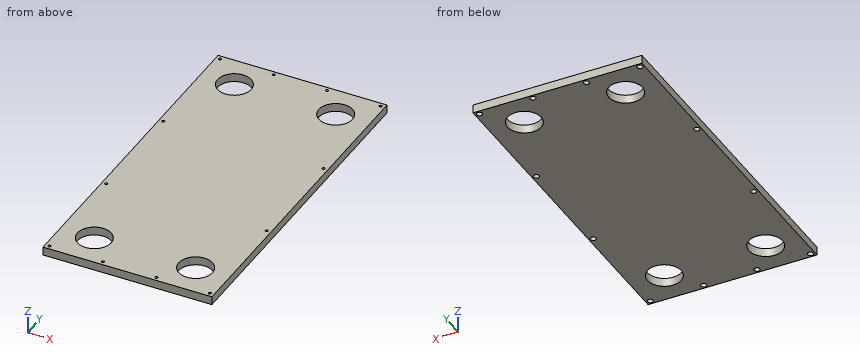
from build123d import *

# Parameters (mm, degrees)
SKETCH1_W                 = 600
SKETCH1_H                 = 1200
BOSS_EXTRUDE1_DEPTH       = 30
SKETCH2_R                 = 60
CUT_EXTRUDE1_DEPTH        = 42
SKETCH3_R                 = 5
CUT_EXTRUDE2_DEPTH        = 40
LPATTERN1_COUNT           = 4
LPATTERN1_PITCH           = 390
LPATTERN2_COUNT           = 2
LPATTERN2_PITCH           = 570
LPATTERN2_COPY_1_SKETCH_R = 5
LPATTERN2_COPY_1_DEPTH    = 40
LPATTERN2_COPY_2_SKETCH_R = 5
LPATTERN2_COPY_2_DEPTH    = 40
LPATTERN2_COPY_3_SKETCH_R = 5
LPATTERN2_COPY_3_DEPTH    = 40
LPATTERN3_COUNT           = 3
LPATTERN3_PITCH           = 190
LPATTERN4_COPY_1_SKETCH_R = 5
LPATTERN4_COPY_1_DEPTH    = 40
LPATTERN4_COPY_2_SKETCH_R = 5
LPATTERN4_COPY_2_DEPTH    = 40
LPATTERN4_COPY_3_SKETCH_R = 5
LPATTERN4_COPY_3_DEPTH    = 40
SKETCH4_R                 = 10
CUT_EXTRUDE3_DEPTH        = 15
LPATTERN5_COUNT           = 4
LPATTERN5_PITCH           = 390
LPATTERN6_COUNT           = 2
LPATTERN6_PITCH           = 570
LPATTERN6_COPY_1_SKETCH_R = 10
LPATTERN6_COPY_1_DEPTH    = 15
LPATTERN6_COPY_2_SKETCH_R = 10
LPATTERN6_COPY_2_DEPTH    = 15
LPATTERN6_COPY_3_SKETCH_R = 10
LPATTERN6_COPY_3_DEPTH    = 15
LPATTERN8_COUNT           = 3
LPATTERN8_PITCH           = 190
LPATTERN9_COPY_1_SKETCH_R = 10
LPATTERN9_COPY_1_DEPTH    = 15
LPATTERN9_COPY_2_SKETCH_R = 10
LPATTERN9_COPY_2_DEPTH    = 15
LPATTERN9_COPY_3_SKETCH_R = 10
LPATTERN9_COPY_3_DEPTH    = 15


with BuildPart() as part:
    # Sketch1 → Boss-Extrude1 (new body)
    with BuildSketch(Plane.XY):
        Rectangle(SKETCH1_W, SKETCH1_H)
    extrude(amount=BOSS_EXTRUDE1_DEPTH)

    # Sketch2 → Cut-Extrude1 (cut)
    with BuildSketch(Plane(origin=(0, 0, 0), x_dir=(-1, 0, 0), z_dir=(0, 0, -1))):
        with Locations((-180, 480)):
            Circle(SKETCH2_R)
        with Locations((180, 480)):
            Circle(SKETCH2_R)
        with Locations((180, -480)):
            Circle(SKETCH2_R)
        with Locations((-180, -480)):
            Circle(SKETCH2_R)
    extrude(amount=-CUT_EXTRUDE1_DEPTH, mode=Mode.SUBTRACT)

    # Sketch3 → Cut-Extrude2 (cut)
    with BuildSketch(Plane(origin=(0, 0, 0), x_dir=(-1, 0, 0), z_dir=(0, 0, -1))):
        with Locations((-285, 585)):
            Circle(SKETCH3_R)
    cut_extrude2 = extrude(amount=-CUT_EXTRUDE2_DEPTH, mode=Mode.SUBTRACT)

    # LPattern1: Cut-Extrude2 ×4
    with Locations(*[(0, -i * LPATTERN1_PITCH, 0) for i in range(1, LPATTERN1_COUNT)]):
        add(cut_extrude2, mode=Mode.SUBTRACT)

    # LPattern2: Cut-Extrude2 ×2
    with Locations(*[(-i * LPATTERN2_PITCH, 0, 0) for i in range(1, LPATTERN2_COUNT)]):
        add(cut_extrude2, mode=Mode.SUBTRACT)

    # LPattern2 copy 1 sketch → LPattern2 copy 1 (cut)
    with BuildSketch(Plane(origin=(-570, -390, 0), x_dir=(-1, 0, 0), z_dir=(0, 0, -1))):
        with Locations((-285, 585)):
            Circle(LPATTERN2_COPY_1_SKETCH_R)
    extrude(amount=-LPATTERN2_COPY_1_DEPTH, mode=Mode.SUBTRACT)

    # LPattern2 copy 2 sketch → LPattern2 copy 2 (cut)
    with BuildSketch(Plane(origin=(-570, -780, 0), x_dir=(-1, 0, 0), z_dir=(0, 0, -1))):
        with Locations((-285, 585)):
            Circle(LPATTERN2_COPY_2_SKETCH_R)
    extrude(amount=-LPATTERN2_COPY_2_DEPTH, mode=Mode.SUBTRACT)

    # LPattern2 copy 3 sketch → LPattern2 copy 3 (cut)
    with BuildSketch(Plane(origin=(-570, -1170, 0), x_dir=(-1, 0, 0), z_dir=(0, 0, -1))):
        with Locations((-285, 585)):
            Circle(LPATTERN2_COPY_3_SKETCH_R)
    extrude(amount=-LPATTERN2_COPY_3_DEPTH, mode=Mode.SUBTRACT)

    # LPattern3: Cut-Extrude2 ×3
    with Locations(*[(-i * LPATTERN3_PITCH, 0, 0) for i in range(1, LPATTERN3_COUNT)]):
        add(cut_extrude2, mode=Mode.SUBTRACT)

    # LPattern4 copy 1 sketch → LPattern4 copy 1 (cut)
    with BuildSketch(Plane(origin=(-190, -1170, 0), x_dir=(-1, 0, 0), z_dir=(0, 0, -1))):
        with Locations((-285, 585)):
            Circle(LPATTERN4_COPY_1_SKETCH_R)
    extrude(amount=-LPATTERN4_COPY_1_DEPTH, mode=Mode.SUBTRACT)

    # LPattern4 copy 2 sketch → LPattern4 copy 2 (cut)
    with BuildSketch(Plane(origin=(-380, -1170, 0), x_dir=(-1, 0, 0), z_dir=(0, 0, -1))):
        with Locations((-285, 585)):
            Circle(LPATTERN4_COPY_2_SKETCH_R)
    extrude(amount=-LPATTERN4_COPY_2_DEPTH, mode=Mode.SUBTRACT)

    # LPattern4 copy 3 sketch → LPattern4 copy 3 (cut)
    with BuildSketch(Plane(origin=(0, -1170, 0), x_dir=(-1, 0, 0), z_dir=(0, 0, -1))):
        with Locations((-285, 585)):
            Circle(LPATTERN4_COPY_3_SKETCH_R)
    extrude(amount=-LPATTERN4_COPY_3_DEPTH, mode=Mode.SUBTRACT)

    # Sketch4 → Cut-Extrude3 (cut)
    with BuildSketch(Plane(origin=(0, 0, 0), x_dir=(-1, 0, 0), z_dir=(0, 0, -1))):
        with Locations((-285, 585)):
            Circle(SKETCH4_R)
    cut_extrude3 = extrude(amount=-CUT_EXTRUDE3_DEPTH, mode=Mode.SUBTRACT)

    # LPattern5: Cut-Extrude3 ×4
    with Locations(*[(0, -i * LPATTERN5_PITCH, 0) for i in range(1, LPATTERN5_COUNT)]):
        add(cut_extrude3, mode=Mode.SUBTRACT)

    # LPattern6: Cut-Extrude3 ×2
    with Locations(*[(-i * LPATTERN6_PITCH, 0, 0) for i in range(1, LPATTERN6_COUNT)]):
        add(cut_extrude3, mode=Mode.SUBTRACT)

    # LPattern6 copy 1 sketch → LPattern6 copy 1 (cut)
    with BuildSketch(Plane(origin=(-570, -390, 0), x_dir=(-1, 0, 0), z_dir=(0, 0, -1))):
        with Locations((-285, 585)):
            Circle(LPATTERN6_COPY_1_SKETCH_R)
    extrude(amount=-LPATTERN6_COPY_1_DEPTH, mode=Mode.SUBTRACT)

    # LPattern6 copy 2 sketch → LPattern6 copy 2 (cut)
    with BuildSketch(Plane(origin=(-570, -780, 0), x_dir=(-1, 0, 0), z_dir=(0, 0, -1))):
        with Locations((-285, 585)):
            Circle(LPATTERN6_COPY_2_SKETCH_R)
    extrude(amount=-LPATTERN6_COPY_2_DEPTH, mode=Mode.SUBTRACT)

    # LPattern6 copy 3 sketch → LPattern6 copy 3 (cut)
    with BuildSketch(Plane(origin=(-570, -1170, 0), x_dir=(-1, 0, 0), z_dir=(0, 0, -1))):
        with Locations((-285, 585)):
            Circle(LPATTERN6_COPY_3_SKETCH_R)
    extrude(amount=-LPATTERN6_COPY_3_DEPTH, mode=Mode.SUBTRACT)

    # LPattern8: Cut-Extrude3 ×3
    with Locations(*[(-i * LPATTERN8_PITCH, 0, 0) for i in range(1, LPATTERN8_COUNT)]):
        add(cut_extrude3, mode=Mode.SUBTRACT)

    # LPattern9 copy 1 sketch → LPattern9 copy 1 (cut)
    with BuildSketch(Plane(origin=(-190, -1170, 0), x_dir=(-1, 0, 0), z_dir=(0, 0, -1))):
        with Locations((-285, 585)):
            Circle(LPATTERN9_COPY_1_SKETCH_R)
    extrude(amount=-LPATTERN9_COPY_1_DEPTH, mode=Mode.SUBTRACT)

    # LPattern9 copy 2 sketch → LPattern9 copy 2 (cut)
    with BuildSketch(Plane(origin=(-380, -1170, 0), x_dir=(-1, 0, 0), z_dir=(0, 0, -1))):
        with Locations((-285, 585)):
            Circle(LPATTERN9_COPY_2_SKETCH_R)
    extrude(amount=-LPATTERN9_COPY_2_DEPTH, mode=Mode.SUBTRACT)

    # LPattern9 copy 3 sketch → LPattern9 copy 3 (cut)
    with BuildSketch(Plane(origin=(0, -1170, 0), x_dir=(-1, 0, 0), z_dir=(0, 0, -1))):
        with Locations((-285, 585)):
            Circle(LPATTERN9_COPY_3_SKETCH_R)
    extrude(amount=-LPATTERN9_COPY_3_DEPTH, mode=Mode.SUBTRACT)


solid = part.part
Could you check a few things on this model? Use its own coordinates, in mm. Give positions to 0.01 mm unless a question says otherwise; leave off trailing zeros. Order: outer loops, then holes, each group sorted by start corner. A loop starts at its lowest first (then second) coordinate and runs counter-clockwise, first axis right, second up. Notation, with made-up numbers: (52.25, 4.25) - (94.25, 4.25) arc R5 cw to (94.25, 13.25) - close; hole circle Ø7 at (84, 62). An arc over 180 degrees is marked (long way). Return JSON: item names as keys, results as strings. Group by question number.
Q1. Suppose I cut it at C-C, the plane x = 209.5. Please give me the cut outline in (y, z), and give its area (3 significant figures).
Q2. Will these pins go through, and if not, where does the flat tip stop? pin 1 Ø10 at (x, y) = (-97.5, -582) entering from -Z; pin 2 Ø23 at (x, y) = (95, -585) entering from -Z.
Q3. Please list where these lines run through material, in increasing order: line 1 along Y through (x, z) = (95, 19.25); line 2 along X through (y, z) = (-585, 11); line 3 along X through (y, z) = (585, 24.5). Write a range as [from, to].
Q4. Suppose I cut it at A-A, the plane y = -480. Please give me the cut outline in (x, z), and give its area (3 significant figures).
Q5. Suppose I cut it at B-B, the plane z = 5.75. State how many separate pieces and enclosed holes the cut face has, and give its area (3 significant figures).
Resolved:
{
 "1": {"outline": "(-600, 0) - (-532.25, 0) - (-532.25, 30) - (-600, 30) - close; (-427.75, 0) - (427.75, 0) - (427.75, 30) - (-427.75, 30) - close; (532.25, 0) - (600, 0) - (600, 30) - (532.25, 30) - close", "area": "29,700 mm2"},
 "2": {"pin 1": "stops at z = 15", "pin 2": "stops at z = 0"},
 "3": {"line 1": "y = [-600, -590], [-580, 580], [590, 600]", "line 2": "x = [-300, -295], [-275, -105], [-85, 85], [105, 275], [295, 300]", "line 3": "x = [-300, -290], [-280, -100], [-90, 90], [100, 280], [290, 300]"},
 "4": {"outline": "(-300, 0) - (-240, 0) - (-240, 30) - (-300, 30) - close; (-120, 0) - (120, 0) - (120, 30) - (-120, 30) - close; (240, 0) - (300, 0) - (300, 30) - (240, 30) - close", "area": "10,800 mm2"},
 "5": {"separate pieces": "1", "enclosed holes": "16", "area": "671,000 mm2"}
}
